```python
from build123d import *

# Parameters (mm, degrees)
SKETCH_1_R            = 5
EXTRUDE_1_DEPTH       = 6
SKETCH_2_R            = 6
EXTRUDE_2_DEPTH       = 6
SKETCH_3_R            = 4.5
EXTRUDE_3_DEPTH       = 20
CHAMFER_1_SIZE        = 0.3
SKETCH_7_W            = 8.670570122
SKETCH_7_H            = 17.253558728
SKETCH_7_W_2          = 11.735923196
CUT_EXTRUDE_1_DEPTH   = 10
HOLE_WIZARD_5_0_5_1_D = 5
SKETCH_8_W            = 3.075789072
SKETCH_8_H            = 1
SKETCH_9_W            = 7.38579235
SKETCH_9_H            = 17.49729378
SKETCH_9_W_2          = 12.485506115
SKETCH_9_H_2          = 24.97101223
CUT_EXTRUDE_2_DEPTH   = 10
CHAMFER_7_SIZE        = 0.3


with BuildPart() as part:
    # 草图1 → 凸台-拉伸1 (new body)
    with BuildSketch(Plane(origin=(0, 0, 0), x_dir=(1, 0, 0), z_dir=(0, 1, 0))):
        with Locations(Location((0, 0, 0), (0, 0, 270))):
            Circle(SKETCH_1_R)
    extrude(amount=-EXTRUDE_1_DEPTH)

    # 草图2 → 凸台-拉伸2 (add)
    with BuildSketch(Plane.XZ.offset(6)):
        with Locations(Location((0, 0, 0), (0, 0, 270))):
            Circle(SKETCH_2_R)
    extrude(amount=EXTRUDE_2_DEPTH)

    # 草图3 → 凸台-拉伸3 (add)
    with BuildSketch(Plane.XZ.offset(12)):
        with Locations(Location((0, 0, 0), (0, 0, 270))):
            Circle(SKETCH_3_R)
    extrude(amount=EXTRUDE_3_DEPTH)

    # 倒角1
    chamfer_1_edges = [part.edges().sort_by_distance(p)[0] for p in [
        (0, 0, -5),
        (0, -6, 6),
        (0, -12, 6),
    ]]
    chamfer(chamfer_1_edges, length=CHAMFER_1_SIZE)

    # 草图7 → 切除-拉伸1 (cut, symmetric)
    with BuildSketch(Plane.XY):
        with Locations((-9.835285061, -4.858845759)):
            Rectangle(SKETCH_7_W, SKETCH_7_H)
        with Locations((11.367961598, -4.858845759)):
            Rectangle(SKETCH_7_W_2, SKETCH_7_H)
    extrude(amount=CUT_EXTRUDE_1_DEPTH, both=True, mode=Mode.SUBTRACT)

    # Ø5.0 (5) 直径孔1 (through all)
    with Locations(Plane(origin=(0, 0, 0), x_dir=(1, 0, 0), z_dir=(0, 1, 0))):
        with Locations((0, 0)):
            Hole(HOLE_WIZARD_5_0_5_1_D / 2)

    # 草图8 → 切除-旋转1 (revolve, cut)
    with BuildSketch(Plane.XY, mode=Mode.PRIVATE) as cut_revolve_1_sk:
        with Locations((-6.037894536, -5.5)):
            Rectangle(SKETCH_8_W, SKETCH_8_H)
    revolve(cut_revolve_1_sk.sketch.rotate(Axis((0, -6, 0), (0, 1, 0)), 270), axis=Axis((0, -6, 0), (0, 1, 0)), mode=Mode.SUBTRACT)

    # 草图9 → 切除-拉伸2 (cut, symmetric)
    with BuildSketch(Plane(origin=(0, 0, 0), x_dir=(0, 0, -1), z_dir=(1, 0, 0))):
        with Locations((-9.192896175, -6.091907364)):
            Rectangle(SKETCH_9_W, SKETCH_9_H)
        with Locations((11.742753057, -3.629976581)):
            Rectangle(SKETCH_9_W_2, SKETCH_9_H_2)
    extrude(amount=CUT_EXTRUDE_2_DEPTH, both=True, mode=Mode.SUBTRACT)

    # 倒角7
    chamfer_7_edges = [part.edges().sort_by_distance(p)[0] for p in [
        (0, -32, 4.5),
    ]]
    chamfer(chamfer_7_edges, length=CHAMFER_7_SIZE)


solid = part.part
```
Model file for the job. Use its own axes, mm. A direction names the side the tool comes from. Coordinates: 2 decimals unless noted, no trailing zeros. Write each loop counter-clockwise with the first axis right and the second up, starting at its lowest first coordinate (ties: lowest second). Pieces come first, ordered by that corner, then holes. Notation, with made-up numbers: (80.25, 43) - (89.25, 43) arc R36 cw to (89.25, 81) - close; hole circle Ø11 at (1, -19.5). An arc over 180 degrees is marked (long way). One line per item, written item: value. Start each with the question number.
1. Tool access for faces 4 (the conical face through (-4.08, -11.89, 4.14)), 5 (the flat face through (0, -12, 5)), 6 (the cylindrical face through (-4.88, -2.62, -1.08)): list every direction of +Z, -Z, +X, -X, +Y, -Y with a clear straight run to the whole face (end or side of a thin tool).
2. Probe line 1 (Z direction, x = 0.75, y = -23.5); line 2 (X direction, y = -17, z = 1.5); line 3 (Z direction, x = -1.25, y = -18). List the from-to ranges inside material, lowest first. Write a range as from..to.
3. Slice it at C-C (y = -13.5). Write the cut outline in (x, z), plus the area to 3 significant figures.
4. Mould opens along Y. For faces 1 (the cylindrical face through (4.22, -8.962, -4.265)), 2 (the conical face through (-4.14, -6.11, -4.08)), 3 (the flat face through (0, -6, 5)) say: released by +Y, released by -Y, zero draft, split by the parting line, or undercut.
5. Slice it at B-B (x = 0). Write the cut outline in (y, z).
6. Flat gauge pins, fed straight in: pin 1 (1 mm diameter, centred on x = 3, y = -18, fed in from +Z); pin 2 (3 mm diameter, centred on y = -28, z = 3, fed in from -X); pin 3 (3 mm diameter, centred on y = -20, z = 0, fed in from +X). Where does each tip first touch, or does it go through?
7. Slice it at A-A (z = 0). Write the cut outline in (x, y), plus the area to 3 significant figures.
Answers below:
1. face 4: +Z, -X, -Y
1. face 5: -Y
1. face 6: +Y
2. line 1: z = -4.44..-2.38, 2.38..4.44
2. line 2: x = -4.24..-2, 2..4.24
2. line 3: z = -4.32..-2.17, 2.17..4.32
3. outline: circle Ø9 at (0, 0); hole circle Ø5 at (0, 0)
3. area: 44.0 mm^2
4. face 1: zero draft
4. face 2: released by +Y
4. face 3: undercut
5. outline: (-32, -4.2) - (-31.7, -4.5) - (-12, -4.5) - (-12, -5.5) - (-6, -5.5) - (-6, -4.5) - (-5, -4.5) - (-5, -5) - (-0.3, -5) - (0, -4.7) - (0, -2.5) - (-32, -2.5) - close; (-32, 2.5) - (0, 2.5) - (0, 4.7) - (-0.3, 5) - (-5, 5) - (-5, 4.5) - (-6, 4.5) - (-6, 5.5) - (-12, 5.5) - (-12, 4.5) - (-31.7, 4.5) - (-32, 4.2) - close
6. pin 1: stops at z = 3.74
6. pin 2: stops at x = -4.24
6. pin 3: stops at x = 4.5
7. outline: (-5.5, -12) - (-4.5, -12) - (-4.5, -31.7) - (-4.2, -32) - (-2.5, -32) - (-2.5, 0) - (-4.7, 0) - (-5, -0.3) - (-5, -5) - (-4.5, -5) - (-4.5, -6) - (-5.5, -6) - close; (2.5, -32) - (4.2, -32) - (4.5, -31.7) - (4.5, -12) - (5.5, -12) - (5.5, -6) - (4.5, -6) - (4.5, -5) - (5, -5) - (5, -0.3) - (4.7, 0) - (2.5, 0) - close
7. area: 145 mm^2
